The listing builds one solid part. Answer for the finished solid, in the listing's coordinates (mm). A direction names the side the tool comes from. Give positions to 0.01 mm unless a question says otherwise; leave off trailing zeros. Write each loop counter-clockwise with the first axis right and the second up, starting at its lowest first coordinate (ties: lowest second). Pieces come first, ordered by that corner, then holes. Notation, with made-up numbers: (-5.5, 65) - (31.5, 65) arc R20 cw to (31.5, 81) - close; hole circle Ø1 at (-8.5, 67.5). An arc over 180 degrees is marked (long way). One line per question, with ' | ' between items. Start each with the question number.
1. A cutting plane is placed at A-A (x = 6). Determine the outline of the cut face in (y, z), then the cut area to 4 significant figures.
2. The mould has two halves that part along Y. Classify faces 1 (the face through (-0.1, 8, -2.2)), 2 (the face through (0.33, 0.32, -7.493)), 3 (the face through (0.1, 5.5, 3.2)), 4 (the face through (2, 0.65, 5)): +Y half, -Y half, draft (parallel to the pull), parting line (faces both ways), or undercut.
3. Given P1, Ø3, axis at y = 6.5, z = -2.5, coming from the +X side; P2, Ø1, axis at y = 4, z = -0.5, coming from the -X side; P3, Ø3, axis at x = -6, y = 1, coming from the +Z side, each flat-ended and moving along its own axis, determine where each tip first touches the part or whether it passes through.
4. A cutting plane is placed at B-B (z = 0). Determine the outline of the cut face in (x, y), then the cut area to 4 significant figures.
5. A cutting plane is placed at D-D (y = 7). Determine the outline of the cut face in (x, z), then the cut area to 3 significant figures.
6. Find the intervals of material crossed by L1, parallel to Y at x = 5.5, z = -4; L2, parallel to X at y = 6.15, z = 0; L3, parallel to X at y = 2.8, z = 0, in increasing order. Write a range as from..to.
7. A cutting plane is placed at C-C (z = -6.5). Determine the outline of the cut face in (x, y), then the cut area to 3 significant figures.
8. For faces 5 (the face through (3.3, 7.3, -0.1)), 6 (the face through (-2, 2, 0)), 7 (the face through (0.33, 5.094, -7.493)), 8 (the face through (4.88, 7.65, 1.08)), 9 (the face through (2, 0, -2)), determine the directions among +Z, -Z, +X, -X, +Y, -Y from which every point of the face is accessible in a straight line to the end or side of a thin tool.
```python
from build123d import *

# Parameters (mm, degrees)
SKETCH1_R           = 7.5
BOSS_EXTRUDE1_DEPTH = 4
SKETCH3_W           = 3
SKETCH3_H           = 3.25
SKETCH4_R           = 5
BOSS_EXTRUDE2_DEPTH = 8
SKETCH5_W           = 2
SKETCH5_H           = 1.8
SKETCH6_R           = 2
CUT_EXTRUDE1_DEPTH  = 14.285330256
CUT_EXTRUDE3_START  = -2
SKETCH7_R           = 8.572097994
SKETCH7_R_2         = 5
CUT_EXTRUDE3_DEPTH  = 2
BOSS_EXTRUDE3_START = -0.8
SKETCH8_R           = 7.5
BOSS_EXTRUDE3_DEPTH = 0.8


with BuildPart() as part:
    # Sketch1 → Boss-Extrude1 (new body)
    with BuildSketch(Plane(origin=(0, 0, 0), x_dir=(1, 0, 0), z_dir=(0, 1, 0))):
        with Locations(Location((0, 0, 0), (0, 0, 270))):
            Circle(SKETCH1_R)
    extrude(amount=BOSS_EXTRUDE1_DEPTH)

    # Sketch3 → Cut-Revolve1 (revolve, cut)
    with BuildSketch(Plane.XY, mode=Mode.PRIVATE) as cut_revolve1_sk:
        with Locations((6, 2.275)):
            Rectangle(SKETCH3_W, SKETCH3_H)
    revolve(cut_revolve1_sk.sketch.rotate(Axis((0, 0, 0), (0, 1, 0)), 90), axis=Axis((0, 0, 0), (0, 1, 0)), mode=Mode.SUBTRACT)

    # Sketch4 → Boss-Extrude2 (add)
    with BuildSketch(Plane(origin=(0, 0, 0), x_dir=(1, 0, 0), z_dir=(0, 1, 0))):
        with Locations(Location((0, 0, 0), (0, 0, 90))):
            Circle(SKETCH4_R)
    extrude(amount=BOSS_EXTRUDE2_DEPTH)

    # Sketch5 → Cut-Revolve2 (revolve, cut)
    with BuildSketch(Plane.XY, mode=Mode.PRIVATE) as cut_revolve2_sk:
        with Locations((4, 6.4)):
            Rectangle(SKETCH5_W, SKETCH5_H)
    revolve(cut_revolve2_sk.sketch.rotate(Axis((0, 4, 0), (0, 1, 0)), 90), axis=Axis((0, 4, 0), (0, 1, 0)), mode=Mode.SUBTRACT)

    # Sketch6 → Cut-Extrude1 (cut, through all)
    with BuildSketch(Plane(origin=(0, 8, 0), x_dir=(1, 0, 0), z_dir=(0, 1, 0))):
        with Locations(Location((0, 0, 0), (0, 0, 270))):
            Circle(SKETCH6_R)
    extrude(amount=-CUT_EXTRUDE1_DEPTH, mode=Mode.SUBTRACT)

    # Sketch7 → Cut-Extrude3 (cut)
    with BuildSketch(Plane(origin=(0, 4, 0), x_dir=(1, 0, 0), z_dir=(0, 1, 0)).offset(CUT_EXTRUDE3_START)):
        Circle(SKETCH7_R)
        with Locations(Location((0, 0, 0), (0, 0, 90))):
            Circle(SKETCH7_R_2, mode=Mode.SUBTRACT)
    extrude(amount=CUT_EXTRUDE3_DEPTH, mode=Mode.SUBTRACT)

    # Sketch8 → Boss-Extrude3 (add)
    with BuildSketch(Plane(origin=(0, 5.5, 0), x_dir=(1, 0, 0), z_dir=(0, 1, 0)).offset(BOSS_EXTRUDE3_START)):
        with Locations(Location((0, 0, 0), (0, 0, 270))):
            Circle(SKETCH8_R)
    extrude(amount=BOSS_EXTRUDE3_DEPTH)


solid = part.part
```
Determined:
1) outline: (0, -4.5) - (0.65, -4.5) - (0.65, 4.5) - (0, 4.5) - close; (4.7, -4.5) - (5.5, -4.5) - (5.5, 4.5) - (4.7, 4.5) - close | area: 13.05 mm2
2) face 1: +Y half | face 2: draft | face 3: undercut | face 4: undercut
3) P1: x = 7.37 | P2: x = -5 | P3: z = 5.97
4) outline: (-7.5, 0) - (-2, 0) - (-2, 4.7) - (2, 4.7) - (2, 0) - (7.5, 0) - (7.5, 0.65) - (5, 0.65) - (5, 4.7) - (7.5, 4.7) - (7.5, 5.5) - (3, 5.5) - (3, 7.3) - (5, 7.3) - (5, 8) - (2, 8) - (2, 5.5) - (-2, 5.5) - (-2, 8) - (-5, 8) - (-5, 7.3) - (-3, 7.3) - (-3, 5.5) - (-7.5, 5.5) - (-7.5, 4.7) - (-5, 4.7) - (-5, 0.65) - (-7.5, 0.65) - close | area: 51.25 mm2
5) outline: circle Ø6 at (0, 0); hole circle Ø4 at (0, 0) | area: 15.7 mm2
6) L1: 0..0.65, 4.7..5.5 | L2: -3..-2, 2..3 | L3: -5..-2, 2..5
7) outline: (-3.74, 0) - (3.74, 0) - (3.74, 0.65) - (-3.74, 0.65) - close; (-3.74, 4.7) - (3.74, 4.7) - (3.74, 5.5) - (-3.74, 5.5) - close | area: 10.9 mm2
8) face 5: none | face 6: -Y | face 7: +Y, -Y | face 8: +Y | face 9: +Z, -Z, +X, -X, -Y
